Verification items for the finished model (mm, model axes). A direction names the side the tool comes from. Give positions to 0.01 mm unless a question says otherwise; leave off trailing zeros. Loops run counter-clockwise (first coordinate to the right, second up) from the corner with the lowest first, then second, coordinate; pieces in that order, holes last. Notation, with made-up numbers: (-23, 6.25) - (-12, 6.25) arc R33 cw to (-12, 37.25) - close; hole circle Ø2 at (38, 79.5). An arc over 180 degrees is marked (long way). Put each result on its own line as item: value. Start each with the question number.
```python
from build123d import *

# Parameters (mm, degrees)
LINK_BLOCK_SKETCH_W               = 46
LINK_BLOCK_SKETCH_H               = 20
LINK_BLOCK_DEPTH                  = 10
FIRST_LUG_PROFILE_SKETCH_R        = 7
FIRST_LUG_PROFILE_BORE_CUT_DEPTH  = 35
SECOND_LUG_PROFILE_SKETCH_W       = 55.121968116
SECOND_LUG_PROFILE_SKETCH_H       = 28.549832612
SECOND_LUG_PROFILE_SKETCH_R       = 7
SECOND_LUG_PROFILE_BORE_CUT_DEPTH = 35


with BuildPart() as part:
    # Link Block Sketch → Link Block (new, symmetric)
    with BuildSketch(Plane.XY):
        Rectangle(LINK_BLOCK_SKETCH_W, LINK_BLOCK_SKETCH_H)
    extrude(amount=LINK_BLOCK_DEPTH, both=True)

    # First Lug Profile Sketch → First Lug Profile & Bore Cut (cut, symmetric)
    with BuildSketch(Plane.XY.offset(10)):
        with BuildLine():
            ThreePointArc((-7.472292016, 8.333333333), (-2.19037874, 5.851457845), (3.583123952, 5))
            Line((3.583123952, 5), (23, 5))
            Line((23, 5), (23, 10))
            Line((23, 10), (-13, 10))
            ThreePointArc((-13, 10), (-10.113248654, 9.574271078), (-7.472292016, 8.333333333))
        make_face()
        with BuildLine():
            ThreePointArc((-23, -4.3e-08), (-20.071067827, 7.071067797), (-13, 10))
            Line((-13, 10), (-23, 10))
            Line((-23, 10), (-23, -4.3e-08))
        make_face()
        with BuildLine():
            ThreePointArc((-13, -10), (-20.071067797, -7.071067827), (-23, -4.3e-08))
            Line((-23, -4.3e-08), (-23, -10))
            Line((-23, -10), (-13, -10))
        make_face()
        with BuildLine():
            Line((23, -10), (23, -5))
            Line((23, -5), (3.583123952, -5))
            ThreePointArc((3.583123952, -5), (-2.19037874, -5.851457845), (-7.472292016, -8.333333333))
            ThreePointArc((-7.472292016, -8.333333333), (-10.113248654, -9.574271078), (-13, -10))
            Line((-13, -10), (23, -10))
        make_face()
        with Locations((-13, 0)):
            Circle(FIRST_LUG_PROFILE_SKETCH_R)
    extrude(amount=FIRST_LUG_PROFILE_BORE_CUT_DEPTH, both=True, mode=Mode.SUBTRACT)

    # Second Lug Profile Sketch → Second Lug Profile & Bore Cut (cut, symmetric)
    # profile 1 of 6: a face of its own
    with BuildSketch(Plane.XZ.offset(5)):
        with Locations((1.394530012, 1.140979101)):
            Rectangle(SECOND_LUG_PROFILE_SKETCH_W, SECOND_LUG_PROFILE_SKETCH_H)
        with BuildLine():
            Line((-23, -5), (-23, 5))
            Line((-23, 5), (-3.583123952, 5))
            ThreePointArc((-3.583123952, 5), (0.06100146, 5.334793416), (3.583123952, 6.327965002))
            Line((3.583123952, 6.327965002), (3.583123952, 10))
            Line((3.583123952, 10), (13, 10))
            Line((13, 10), (23, 10))
            Line((23, 10), (23, -6e-08))
            Line((23, -6e-08), (23, -10))
            Line((23, -10), (12.999999984, -10))
            Line((12.999999984, -10), (3.583123952, -10))
            Line((3.583123952, -10), (3.583123952, -6.327965002))
            ThreePointArc((3.583123952, -6.327965002), (0.06100146, -5.334793416), (-3.583123952, -5))
            Line((-3.583123952, -5), (-23, -5))
        make_face(mode=Mode.SUBTRACT)
    # profile 2 of 6: a face of its own
    with BuildSketch(Plane.XZ.offset(5)):
        with Locations((13, 0)):
            Circle(SECOND_LUG_PROFILE_SKETCH_R)
    # profile 3 of 6: a face of its own
    with BuildSketch(Plane.XZ.offset(5)):
        with BuildLine():
            Line((23, -10), (23, -6e-08))
            ThreePointArc((23, -6e-08), (20.071067785, -7.071067839), (12.999999984, -10))
            Line((12.999999984, -10), (23, -10))
        make_face()
    # profile 4 of 6: a face of its own
    with BuildSketch(Plane.XZ.offset(5)):
        with BuildLine():
            ThreePointArc((7.472292016, -8.333333333), (5.582716659, -7.223966531), (3.583123952, -6.327965002))
            Line((3.583123952, -6.327965002), (3.583123952, -10))
            Line((3.583123952, -10), (12.999999984, -10))
            ThreePointArc((12.999999984, -10), (10.113248646, -9.574271075), (7.472292016, -8.333333333))
        make_face()
    # profile 5 of 6: a face of its own
    with BuildSketch(Plane.XZ.offset(5)):
        with BuildLine():
            Line((3.583123952, 10), (3.583123952, 6.327965002))
            ThreePointArc((3.583123952, 6.327965002), (5.582716659, 7.223966531), (7.472292016, 8.333333333))
            ThreePointArc((7.472292016, 8.333333333), (10.113248654, 9.574271078), (13, 10))
            Line((13, 10), (3.583123952, 10))
        make_face()
    # profile 6 of 6: a face of its own
    with BuildSketch(Plane.XZ.offset(5)):
        with BuildLine():
            Line((23, 10), (13, 10))
            ThreePointArc((13, 10), (20.071067833, 7.071067791), (23, -6e-08))
            Line((23, -6e-08), (23, 10))
        make_face()
    extrude(amount=SECOND_LUG_PROFILE_BORE_CUT_DEPTH, both=True, mode=Mode.SUBTRACT)


solid = part.part
```
1) Draft check along X on faces 5 (the face through (-11, -7, 5)), 6 (the face through (-2.112, -5.828, -0.089)), 7 (the face through (-20, 0, 0)). Enter one of: pulls with the +X half, pulls with the -X half, needs draft (parallel to the pull), parting line crosses it, or undercut.
2) Section check B-B, the plane z = 2.5. Enter the section's corners in (x, y), plus the area to 3 significant figures.
3) Section check C-C, the plane x = -14.5. Enter the section's corners in (y, z).
4) Section check A-A, the plane y = -0.75. Enter the section's corners in (x, z).
5) Set-up check for faces 1 (the face through (16.23, -0.07, -6.21)), 2 (the face through (-11, -7, -5)), 3 (the face through (11, 5, -7)), 4 (the face through (11, -5, -7)): record each of +Z, -Z, +X, -X, +Y, -Y from which the full face is reachable in a straight line by a thin tool's end or side.
6) Section check D-D, the plane y = 4. Enter the section's corners in (x, z), plus the area to 3 significant figures.
7) Scan lines: line 1 along X through (y, z) = (4, -3.25); line 2 along Y through (x, z) = (-13, 2.75); line 3 along X through (y, z) = (0, -1.5). Record each from-to range of solid material in increasing order. Write a range as from..to.
8) Depth check by flat-ended pin: P1, Ø1.5, axis at x = -14, z = -5, coming from the +Y side; P2, Ø8, axis at y = -5, z = -3.5, coming from the -X side; P3, Ø5, axis at x = 11, z = 6.5, coming from the +Y side. Enter the tip coordinate at first touch or a pass-through.
Results are:
1. face 5: needs draft
1. face 6: pulls with the +X half
1. face 7: undercut
2. outline: (-7.47, -8.33) arc R20 cw to (3.58, -5) - (6.46, -5) - (6.46, 5) - (3.58, 5) arc R20 cw to (-7.47, 8.33) arc R10 ccw (long way) to start; (19.54, -5) - (22.68, -5) - (22.68, 5) - (19.54, 5) - close; hole circle Ø14 at (-13, 0)
2. area: 302 mm2
3. outline: (-9.89, -5) - (-6.84, -5) - (-6.84, 5) - (-9.89, 5) - close; (6.84, -5) - (9.89, -5) - (9.89, 5) - (6.84, 5) - close
4. outline: (-22.97, -5) - (-19.96, -5) - (-19.96, 5) - (-22.97, 5) - close; (-6.04, -5) - (-3.58, -5) arc R20 cw to (7.47, -8.33) arc R10 ccw (long way) to (7.47, 8.33) arc R20 cw to (-3.58, 5) - (-6.04, 5) - close; hole circle Ø14 at (13, 0)
5. face 1: +Y, -Y
5. face 2: -Z, -X, +Y, -Y
5. face 3: +Z, -Z, +X, +Y
5. face 4: +Z, -Z, +X, -Y
6. outline: (-22.17, -5) - (-18.74, -5) - (-18.74, 5) - (-22.17, 5) - close; (-7.26, -5) - (-3.58, -5) arc R20 cw to (7.47, -8.33) arc R10 ccw (long way) to (7.47, 8.33) arc R20 cw to (-3.58, 5) - (-7.26, 5) - close; hole circle Ø14 at (13, 0)
6. area: 313 mm2
7. line 1: x = -22.17..-18.74, -7.26..6.8, 19.2..22.46
7. line 2: y = -10..-7, 7..10
7. line 3: x = -23..-20, -6..6.16, 19.84..22.89
8. P1: stops at y = 10
8. P2: stops at x = -22.95
8. P3: stops at y = 5
